Verification items for the finished model (mm, model axes). A direction names the side the tool comes from. Coordinates: 2 decimals unless noted, no trailing zeros. Order: outer loops, then holes, each group sorted by start corner. A loop starts at its lowest first (then second) coordinate and runs counter-clockwise, first axis right, second up.
Q1. Cross-section at B-B, the plane y = 14. Record the boundary of the cut face in (x, z).
Q2. Depth check by flat-ended pin: P1, Ø10, axis at x = 26, z = -17.5, coming from the -Y side; P2, Ø3, axis at x = 19.5, z = -29, coming from the +Y side; P3, Ø5.5, axis at x = 0, y = -41, coming from the -Z side. Enter the tip coordinate at first touch or a pass-through.
Q3. Cross-section at A-A, the plane z = -32. Record the boundary of the cut face in (x, y).
Q4. Set-up check for faces 1 (the cylindrical face through (-47.69, -15.02, -23.8)), 2 (the cylindrical face through (-44.14, -1.3, -10.01)), 3 (the flat face through (15, 30, -48)), 4 (the cylindrical face through (44.14, -1.3, -37.99)), 5 (the flat face through (-15, 30, 0)): record each of +Z, -Z, +X, -X, +Y, -Y from which the full face is reachable in a straight line by a thin tool's end or side.
Q5. Thickness scan on line 1 (X direction, y = 0, z = -4); line 2 (Z direction, x = 12, y = -54.5); line 3 (Y direction, x = 0, z = -13.5). Record the ranges inside material, lowest first.
Q6. Draft check along Y on faces 6 (the conical face through (-41.317, 0.498, -26.562)), 7 (the flat face through (48, -17, -38)), 8 (the cylindrical face through (55.55, 42.594, -42.93)). Enter one of: pulls with the +Y half, pulls with the -Y half, needs draft (parallel to the pull), parting line crosses it, or undercut.
from build123d import *

# Parameters (mm, degrees)
HOLE_WIZARD_M8_1_D     = 6.8
HOLE_WIZARD_M8_1_DEPTH = 19.75
HOLE_WIZARD_M8_1_TIP   = 2.042926105
HOLE_WIZARD_M8_3_D     = 6.8
HOLE_WIZARD_M8_3_DEPTH = 19.75
HOLE_WIZARD_M8_3_TIP   = 2.042926105


with BuildPart() as part:
    # 草图1 → 旋转1 (revolve)
    with BuildSketch(Plane(origin=(0, 0, 0), x_dir=(1, 0, 0), z_dir=(0, 1, 0))):
        Polygon((-32, 48), (-70, 48), (-70, 38), (-50, 38), (-50, 10), (-70, 10), (-70, 0), (-32, 0), align=None)
    revolve(axis=Axis((0, 0, 0), (0, 0, 1)))

    # M8 螺纹孔1
    with Locations(Plane(origin=(0, 0, -48), x_dir=(-1, 0, 0), z_dir=(0, 0, -1))):
        with Locations((0, 41), (41, 0), (-41, 0), (0, -41)):
            Hole(HOLE_WIZARD_M8_1_D / 2, depth=HOLE_WIZARD_M8_1_DEPTH)
            with Locations((0, 0, -(HOLE_WIZARD_M8_1_DEPTH + HOLE_WIZARD_M8_1_TIP / 2))):  # 118° drill point
                Cone(0, HOLE_WIZARD_M8_1_D / 2, HOLE_WIZARD_M8_1_TIP, mode=Mode.SUBTRACT)

    # M8 螺纹孔3
    with Locations(Plane.XY):
        with Locations((41, 0), (0, -41), (-41, 0), (0, 41)):
            Hole(HOLE_WIZARD_M8_3_D / 2, depth=HOLE_WIZARD_M8_3_DEPTH)
            with Locations((0, 0, -(HOLE_WIZARD_M8_3_DEPTH + HOLE_WIZARD_M8_3_TIP / 2))):  # 118° drill point
                Cone(0, HOLE_WIZARD_M8_3_D / 2, HOLE_WIZARD_M8_3_TIP, mode=Mode.SUBTRACT)


solid = part.part
Check values:
1. outline: (-68.59, -48) - (-28.77, -48) - (-28.77, 0) - (-68.59, 0) - (-68.59, -10) - (-48, -10) - (-48, -38) - (-68.59, -38) - close; (28.77, -48) - (68.59, -48) - (68.59, -38) - (48, -38) - (48, -10) - (68.59, -10) - (68.59, 0) - (28.77, 0) - close
2. P1: stops at y = -45.38
2. P2: stops at y = 46.65
2. P3: stops at z = -27.86
3. outline: circle Ø100 at (0, 0); hole circle Ø6.8 at (-41, 0); hole circle Ø64 at (0, 0); hole circle Ø6.8 at (0, -41); hole circle Ø6.8 at (0, 41); hole circle Ø6.8 at (41, 0)
4. face 1: none
4. face 2: +Z
4. face 3: -Z, +X, -X, +Y, -Y
4. face 4: -Z
4. face 5: +Z, +X, -X, +Y, -Y
5. line 1: x = -70 to -44.4, -37.6 to -32, 32 to 37.6, 44.4 to 70
5. line 2: z = -48 to -38, -10 to 0
5. line 3: y = -50 to -44.4, -37.6 to -32, 32 to 37.6, 44.4 to 50
6. face 6: undercut
6. face 7: needs draft
6. face 8: parting line crosses it
